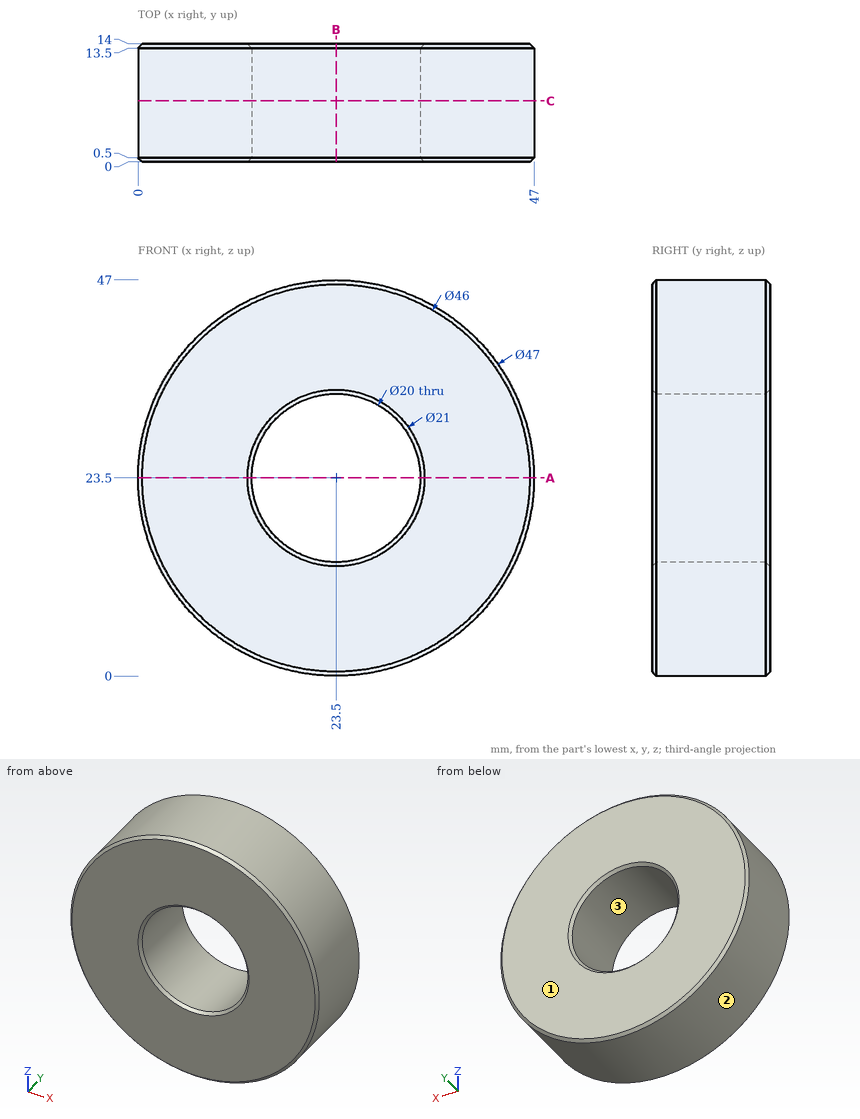
Verification items for this drawing (mm, ordinates from the low corner). Coordinates: 2 decimals unless noted, no trailing zeros. Write each loop counter-clockwise with the first axis right and the second up, starting at its lowest first coordinate (ties: lowest second). Pieces come first, ordered by that corner, then holes. Notation, with made-up numbers: (41.25, 74) -> (90.25, 74) arc R21 ccw to (90.25, 108) -> close; hole circle Ø2 at (25.25, 4). An arc over 180 degrees is marked (long way). One line per item, written item: value. Start each with the question number.
Q1. Mould release check, pull along X, two halves, no side actions. Record for the marked faces 1, 2 and 3: pulls with the +X half, pulls with the -X half, needs draft (parallel to the pull), parting line crosses it, or undercut.
Q2. Cross-section at A-A on z = 23.5. Enter the section's corners in (x, y), and give its area (3 significant figures).
Q3. Cross-section at C-C on y = 7.25. Enter the section's corners in (x, z), and give its area (3 significant figures).
Q4. Thickness scan on L1, parallel to X at y = 6, z = 23.5; L2, parallel to X at y = 9.25, z = 16; L3, parallel to Z at x = 14.5, y = 8. Record the ranges inside material, lowest first. Write a range as from..to.
Q5. Go/stop test with flat-tipped pins: P1, Ø3, axis at x = 5, y = 9.5, coming from the -Z side (3 decimals); P2, Ø1.5, axis at y = 6.5, z = 21.5, coming from the -X side; P3, Ø5, axis at x = 38.5, y = 4.5, coming from the +Z side; P4, Ø12, axis at x = 23.5, z = 23.5, coming from the +Y side. Record where each tip stops, or that it passes through.
Q6. Cross-section at B-B on x = 23.5. Enter the section's corners in (y, z), and give its area (3 significant figures).
Checked values:
1. face 1: needs draft
1. face 2: parting line crosses it
1. face 3: undercut
2. outline: (0, 0.5) -> (0.5, 0) -> (13, 0) -> (13.5, 0.5) -> (13.5, 13.5) -> (13, 14) -> (0.5, 14) -> (0, 13.5) -> close; (33.5, 0.5) -> (34, 0) -> (46.5, 0) -> (47, 0.5) -> (47, 13.5) -> (46.5, 14) -> (34, 14) -> (33.5, 13.5) -> close
2. area: 377 mm²
3. outline: circle Ø47 at (23.5, 23.5); hole circle Ø20 at (23.5, 23.5)
3. area: 1,420 mm²
4. L1: x = 0..13.5, 33.5..47
4. L2: x = 1.23..16.89, 30.11..45.77
4. L3: z = 1.79..19.14, 27.86..45.21
5. P1: stops at z = 7.275
5. P2: stops at x = 0.03
5. P3: stops at z = 43.4
5. P4: passes through
6. outline: (0, 0.5) -> (0.5, 0) -> (13.5, 0) -> (14, 0.5) -> (14, 13) -> (13.5, 13.5) -> (0.5, 13.5) -> (0, 13) -> close; (0, 34) -> (0.5, 33.5) -> (13.5, 33.5) -> (14, 34) -> (14, 46.5) -> (13.5, 47) -> (0.5, 47) -> (0, 46.5) -> close
6. area: 377 mm²
